from build123d import *

# Parameters (mm, degrees)
SKETCH1_W                   = 270
SKETCH1_H                   = 220
SKETCH1_W_2                 = 210
SKETCH1_H_2                 = 160
BOSS_EXTRUDE1_DEPTH         = 30
M8_TAPPED_HOLE1_D           = 6.8
M8_TAPPED_HOLE1_DEPTH       = 21.707073895
M8_TAPPED_HOLE1_CSINK_D     = 8.05
M8_TAPPED_HOLE1_CSINK_ANGLE = 90
M8_TAPPED_HOLE1_TIP         = 2.042926105


with BuildPart() as part:
    # Sketch1 → Boss-Extrude1 (new body)
    with BuildSketch(Plane(origin=(0, 0, 0), x_dir=(1, 0, 0), z_dir=(0, 1, 0))):
        Rectangle(SKETCH1_W, SKETCH1_H)
        Rectangle(SKETCH1_W_2, SKETCH1_H_2, mode=Mode.SUBTRACT)
    extrude(amount=BOSS_EXTRUDE1_DEPTH)

    # M8 Tapped Hole1
    with Locations(Plane(origin=(0, 30, 0), x_dir=(1, 0, 0), z_dir=(0, 1, 0))):
        with Locations((0, 95), (-120, 95), (-120, 0), (-120, -95), (0, -95), (120, -95), (120, 95), (120, 0)):
            CounterSinkHole(M8_TAPPED_HOLE1_D / 2, M8_TAPPED_HOLE1_CSINK_D / 2, depth=M8_TAPPED_HOLE1_DEPTH, counter_sink_angle=M8_TAPPED_HOLE1_CSINK_ANGLE)
            with Locations((0, 0, -(M8_TAPPED_HOLE1_DEPTH + M8_TAPPED_HOLE1_TIP / 2))):  # 118° drill point
                Cone(0, M8_TAPPED_HOLE1_D / 2, M8_TAPPED_HOLE1_TIP, mode=Mode.SUBTRACT)


solid = part.part
Check sheet for the modelled part. Datum: model origin and axes. Units: mm. A direction names the side the tool comes from. Give positions to 0.01 mm unless a question says otherwise; leave off trailing zeros. Write each loop counter-clockwise with the first axis right and the second up, starting at its lowest first coordinate (ties: lowest second). Pieces come first, ordered by that corner, then holes. Notation, with made-up numbers: (-13.5, 66) -> (-1.5, 66) arc R19 ccw to (-1.5, 74) -> close; hole circle Ø3 at (65, 86). An arc over 180 degrees is marked (long way). Use one line per item in the form item = value. Start each with the question number.
1. Section check B-B (x = 48). Record the cut outline in (y, z), and give its area (3 significant figures).
2. Thickness scan on line 1 along X through (y, z) = (12.75, 95); line 2 along Z through (x, y) = (120, 22); line 3 along Z through (x, y) = (0, 12.5). Record the ranges inside material, lowest first. Write a range as from..to.
3. Mould release check, pull along X, two halves, no side actions. Record for faces 4 (the flat face through (-31, 30, 81)), 5 (the flat face through (-135, 15, 2)), 6 (the cylindrical face through (-116.6, 18.7, -0.1)): pulls with the +X half, pulls with the -X half, needs draft (parallel to the pull), parting line crosses it, or undercut.
4. Section check C-C (y = 18.25). Count the separate pieces of the cut face and the enclosed holes in it, and give its area (3 significant figures).
5. Go/stop test with flat-tipped pins: P1, Ø6, axis at x = 0, z = -95, coming from the +Y side; P2, Ø8, axis at x = -120, z = 0, coming from the +Y side (3 decimals). Record where each tip stops, or that it passes through.
6. Section check A-A (z = -72). Record the cut outline in (x, y), and give its area (3 significant figures).
7. Access from +Z, -Z, +X, -X, +Y, -Y to the whole of each face (thin tool, end or side, straight path). Record for faces 1 (the flat face through (-1, 15, 80)), 2 (the flat face through (-2, 15, 110)), 3 (the cylindrical face through (123.4, 18.7, -0.1)).
Conclusion:
q1.outline = (0, -110) -> (30, -110) -> (30, -80) -> (0, -80) -> close; (0, 80) -> (30, 80) -> (30, 110) -> (0, 110) -> close
q1.area = 1,800 mm²
q2.line_1 = -135..-123.4, -116.6..-3.4, 3.4..116.6, 123.4..135
q2.line_2 = -110..-98.4, -91.6..-3.4, 3.4..91.6, 98.4..110
q2.line_3 = -110..-98.4, -91.6..-80, 80..91.6, 98.4..110
q3.face_4 = needs draft
q3.face_5 = pulls with the -X half
q3.face_6 = undercut
q4.separate_pieces = 1
q4.enclosed_holes = 9
q4.area = 25,500 mm²
q5.P1 = 8.05
q5.P2 = 29.975
q6.outline = (-135, 0) -> (-105, 0) -> (-105, 30) -> (-135, 30) -> close; (105, 0) -> (135, 0) -> (135, 30) -> (105, 30) -> close
q6.area = 1,800 mm²
q7.face_1 = +Y, -Y
q7.face_2 = +Z, +X, -X, +Y, -Y
q7.face_3 = +Y
